Can you work these out from the model? Positions are in its coordinate system, mm. Give positions to 0.01 mm unless a question says otherwise; leave off trailing zeros. Loops run counter-clockwise (first coordinate to the right, second up) from the corner with the lowest first, then second, coordinate; pieces in that order, holes last. Notation, with made-up numbers: M 53,73 L 95,73 A18 ccw 95,89 Z; hole C 13.25,88 d7. An arc over 180 degrees is marked long. Use CSV: the item, a comma, the result in double quotes.
from build123d import *

# Parameters (mm, degrees)
SKETCH_1_W          = 310
SKETCH_1_H          = 240
EXTRUDE_1_DEPTH     = 10
SKETCH_2_R          = 13.5
CUT_EXTRUDE_1_DEPTH = 10


with BuildPart() as part:
    # 草图1 → 凸台-拉伸1 (new body)
    with BuildSketch(Plane.XY):
        Rectangle(SKETCH_1_W, SKETCH_1_H)
    extrude(amount=EXTRUDE_1_DEPTH)

    # 草图2 → 切除-拉伸1 (cut)
    with BuildSketch(Plane.XY.offset(10)):
        with Locations((-115, -45)):
            Circle(SKETCH_2_R)
        with Locations((-115, 45)):
            Circle(SKETCH_2_R)
        Polygon((-155, -80), (-45, -120), (-155, -120), align=None)
        Polygon((-155, 80), (-45, 120), (-155, 120), align=None)
    extrude(amount=-CUT_EXTRUDE_1_DEPTH, mode=Mode.SUBTRACT)


solid = part.part
Q1. Please list where these lines run through material, in increasing order: L1, parallel to Y at x = -115, z = 8; L2, parallel to Y at x = -106, z = 1; L3, parallel to X at y = 39, z = 4.5. Write a range as from..to.
Model answer:
L1,"-94.55..-58.5, -31.5..31.5, 58.5..94.55"
L2,"-97.82..-55.06, -34.94..34.94, 55.06..97.82"
L3,"-155..-127.09, -102.91..155"
Q2. I want a section at C-C, the plane x = -115. Please give me the cut outline in (y, z).
Model answer:
outline,"M -94.55,0 L -58.5,0 L -58.5,10 L -94.55,10 Z; M -31.5,0 L 31.5,0 L 31.5,10 L -31.5,10 Z; M 58.5,0 L 94.55,0 L 94.55,10 L 58.5,10 Z"
Q3. I want a section at D-D, the plane y = -90. Please give me the cut outline in (x, z).
Model answer:
outline,"M -127.5,0 L 155,0 L 155,10 L -127.5,10 Z"
Q4. If we mould it in two halves opening along X, with no side actions, what happens to faces 1 (the flat face through (-100.77, 99.72, 5.07)), 2 (the cylindrical face through (-124.95, -35.876, 5.07)), 3 (the flat face through (54, 120, 5))? For each: released by +X, released by -X, zero draft, split by the parting line, or undercut.
Model answer:
face 1,"released by -X"
face 2,"undercut"
face 3,"zero draft"
Q5. I want a section at A-A, the plane y = -45. Please give me the cut outline in (x, z).
Model answer:
outline,"M -155,0 L -128.5,0 L -128.5,10 L -155,10 Z; M -101.5,0 L 155,0 L 155,10 L -101.5,10 Z"
Q6. I'm going to push a flat-ended pin straight in: P1, Ø1, axis at x = -101.5, z = 1.5, coming from the -Y side. Where does the tip first touch, or does it pass through?
Model answer:
P1,"y = -99.64"
Q7. I want a section at B-B, the plane z = 2.75. Please give me the cut outline in (x, y), then the cut area to 3 significant figures.
Model answer:
outline,"M -155,-80 L -45,-120 L 155,-120 L 155,120 L -45,120 L -155,80 Z; hole C -115,-45 d27; hole C -115,45 d27"
area,"68,900 mm2"
